```python
from build123d import *

# Parameters (mm, degrees)
SKETCH1_W           = 1000
SKETCH1_H           = 1500
BOSS_EXTRUDE1_DEPTH = 600
CHAMFER1_SIZE       = 200


with BuildPart() as part:
    # Sketch1 → Boss-Extrude1 (new body)
    with BuildSketch(Plane.XY):
        Rectangle(SKETCH1_W, SKETCH1_H)
    extrude(amount=BOSS_EXTRUDE1_DEPTH)

    # Chamfer1
    chamfer1_edges = [part.edges().sort_by_distance(p)[0] for p in [
        (500, 750, 300),
    ]]
    chamfer(chamfer1_edges, length=CHAMFER1_SIZE)


solid = part.part
```
The listing builds one solid part. Answer for the finished solid, in the listing's coordinates (mm). Coordinates: 2 decimals unless noted, no trailing zeros. Write each loop counter-clockwise with the first axis right and the second up, starting at its lowest first coordinate (ties: lowest second). Pieces come first, ordered by that corner, then holes. Notation, with made-up numbers: (-33, -30.75) - (-4, -30.75) arc R19 cw to (-4, -16.75) - close; hole circle Ø6 at (18, -35). An arc over 180 degrees is marked (long way). Return JSON: item names as keys, results as strings. Group by question number.
Q1. Find the intervals of material crossed by line 1 along X through (y, z) = (570, 111.5); line 2 along Y through (x, z) = (327, 198); line 3 along Y through (x, z) = (414, 417.5), in increasing order. Write a range as [from, to].
Q2. Flat-ended cylindrical pins translate along their axes: pin 1 Ø4 at (x, y) = (177, 403.5) entering from -Z; pin 2 Ø6 at (x, z) = (305.5, 406) entering from +Y. Find the tip coordinate at first contact, or state that the pin passes through.
Q3. The part is cut by section A-A on y = 600. Write down the section's boundary in (x, z).
Evaluation:
{
 "1": {"line 1": "x = [-500, 480]", "line 2": "y = [-750, 723]", "line 3": "y = [-750, 636]"},
 "2": {"pin 1": "stops at z = 0", "pin 2": "stops at y = 747.5"},
 "3": {"outline": "(-500, 0) - (450, 0) - (450, 600) - (-500, 600) - close"}
}
